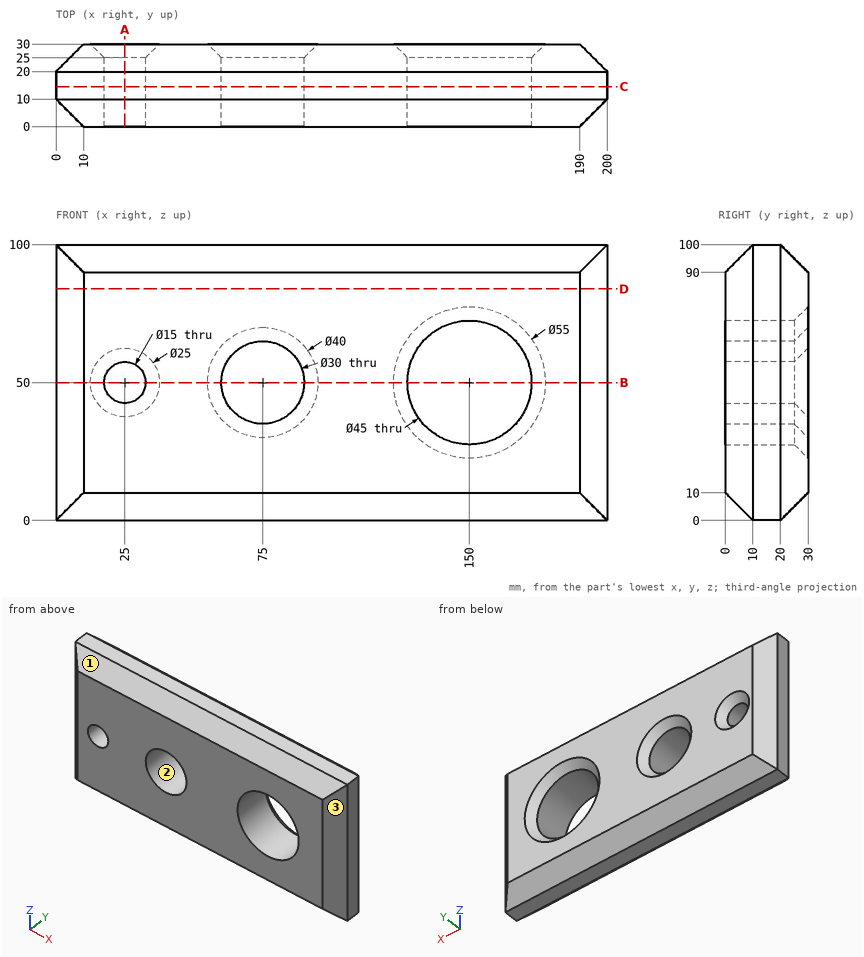
Source: three-view drawing plus pictorial views. Frame: mm from the lowest corner of the part. Round coordinates to 2 decimals unless told otherwise and drop trailing zeros. Loops run counter-clockwise (first coordinate to the right, second up) from the corner with the lowest first, then second, coordinate; pieces in that order, holes last.
Q1. Ray query, line 1 (X direction, y = 7, z = 50); line 2 (X direction, y = 12, z = 61); line 3 (X direction, y = 6.5, z = 48). Return the intervals inside material, ascending.
Q2. Section D-D, the plane z = 84. Return loops of the section in (x, y).
Q3. Section B-B, the plane z = 50. Return loops of the section in (x, y).
Q4. Mould query, pull axis Z, two halves, no side actions, for the marked faces 1, 2 and 3. Classes: pulls with the +Z half, pulls with the -Z half, needs draft (parallel to the pull), parting line crosses it, or undercut.
Q5. Section C-C, the plane y = 14.5. Return loops of the section in (x, z), plus the area to 3 significant figures.
Q6. Section A-A, the plane x = 25. Return loops of the section in (y, z).
Q7. First-contact query: P1, Ø24, axis at x = 25, z = 50, coming from the -Y side; P2, Ø8, axis at x = 100, y = 26, coming from the +Z side; P3, Ø4, axis at x = 45.5, y = 5.5, coming from the +Z side. Flat tips, straight axial feed; report the tip coordinate or a pass-through.
Solutions:
1. line 1: x = 3 to 17.5, 32.5 to 60, 90 to 127.5, 172.5 to 197
1. line 2: x = 0 to 64.8, 85.2 to 130.37, 169.63 to 200
1. line 3: x = 3.5 to 17.77, 32.23 to 60.13, 89.87 to 127.59, 172.41 to 196.5
2. outline: (0, 10) - (10, 0) - (190, 0) - (200, 10) - (200, 20) - (190, 30) - (10, 30) - (0, 20) - close
3. outline: (0, 10) - (10, 0) - (17.5, 0) - (17.5, 25) - (12.5, 30) - (10, 30) - (0, 20) - close; (32.5, 0) - (60, 0) - (60, 25) - (55, 30) - (37.5, 30) - (32.5, 25) - close; (90, 0) - (127.5, 0) - (127.5, 25) - (122.5, 30) - (95, 30) - (90, 25) - close; (172.5, 0) - (190, 0) - (200, 10) - (200, 20) - (190, 30) - (177.5, 30) - (172.5, 25) - close
4. face 1: pulls with the +Z half
4. face 2: undercut
4. face 3: needs draft
5. outline: (0, 0) - (200, 0) - (200, 100) - (0, 100) - close; hole circle Ø15 at (25, 50); hole circle Ø30 at (75, 50); hole circle Ø45 at (150, 50)
5. area: 17,500 mm2
6. outline: (0, 10) - (10, 0) - (20, 0) - (30, 10) - (30, 37.5) - (25, 42.5) - (0, 42.5) - close; (0, 57.5) - (25, 57.5) - (30, 62.5) - (30, 90) - (20, 100) - (10, 100) - (0, 90) - close
7. P1: stops at y = 0
7. P2: stops at z = 98
7. P3: stops at z = 97.5
